For this review, take the finished solid that the model builds, in its own axes (mm). Face numbers are marked on the shaded views. A direction names the side the tool comes from. Round coordinates to 2 decimals unless told otherwise and drop trailing zeros. Loops run counter-clockwise (first coordinate to the right, second up) from the corner with the lowest first, then second, coordinate; pieces in that order, holes last. Notation, with made-up numbers: (75, 30.25) -> (133, 30.25) arc R9 ccw to (133, 38.25) -> close; hole circle Ø1 at (-35, 39.25). An arc over 180 degrees is marked (long way). One line per question, with ' | ' between items. Start each with the question number.
1. For the marked faces 1, 2 and 3, list the 3-axis set-ups (+Z, -Z, +X, -X, +Y, -Y) from which the entire face can be reached by the end or side of a thin tool; tool diameter is ignored.
2. Consider section A-A (y = 0). Write out the cut boundary in (x, z), and give its area (3 significant figures).
3. Consider section C-C (z = 233.5). Write out the cut boundary in (x, y).
4. For pin 1 Ø2.5 at (y, z) = (17.5, -3) entering from -X; pin 2 Ø4 at (y, z) = (26.5, 215.5) entering from +X (3 decimals); pin 3 Ø1 at (x, z) = (23.5, 280) entering from -Y, all flat-tipped, find the tip position at first contact; note any pin that passes through.
5. Wall thickness on line 1 along X through (y, z) = (19.5, 253); line 2 along Y through (x, z) = (-28, 194); line 3 along Z through (x, y) = (28, 15): over which ranges is each line inside the solid? List them lowest first.
6. Consider section B-B (x = 0). Write out the cut boundary in (y, z).
7. Consider section D-D (z = 160.5). Write out the cut boundary in (x, y).
```python
from build123d import *

# Parameters (mm, degrees)
BOSS_EXTRUDE1_DEPTH      = 400
BOSS_EXTRUDE1_DEPTH_BACK = 20
SKETCH1_R                = 25
CHAMFER1_SIZE            = 4
CUT_EXTRUDE1_DEPTH       = 10
SKETCH3_R                = 35
BOSS_EXTRUDE2_DEPTH      = 70
CHAMFER2_SIZE            = 2
CHAMFER3_SIZE            = 4


with BuildPart() as part:
    # Sketch1 → Boss-Extrude1 (new, two sides: drawn at the far end of the back side and taken through both)
    with BuildSketch(Plane.XY.offset(-BOSS_EXTRUDE1_DEPTH_BACK)):
        Circle(SKETCH1_R)
    extrude(amount=BOSS_EXTRUDE1_DEPTH + BOSS_EXTRUDE1_DEPTH_BACK)

    # Chamfer1
    chamfer1_edges = [part.edges().sort_by_distance(p)[0] for p in [
        (-25, 0, -20),
        (-25, 0, 400),
    ]]
    chamfer(chamfer1_edges, length=CHAMFER1_SIZE)

    # Sketch2 → Cut-Extrude1 (cut)
    with BuildSketch(Plane(origin=(0, 25, 0), x_dir=(1, 0, 0), z_dir=(0, 1, 0))):
        with BuildLine():
            Line((7.5, -15), (7.5, 55))
            Line((7.5, 55), (-7.5, 55))
            Line((-7.5, 55), (-7.5, -15))
            ThreePointArc((-7.5, -15), (0, -22.5), (7.5, -15))
        make_face()
    extrude(amount=-CUT_EXTRUDE1_DEPTH, mode=Mode.SUBTRACT)

    # Sketch3 → Boss-Extrude2 (add, symmetric)
    with BuildSketch(Plane.XY.offset(250)):
        Circle(SKETCH3_R)
    extrude(amount=BOSS_EXTRUDE2_DEPTH, both=True)

    # Chamfer2
    chamfer2_edges = [part.edges().sort_by_distance(p)[0] for p in [
        (-35, 0, 180),
        (-35, 0, 320),
    ]]
    chamfer(chamfer2_edges, length=CHAMFER2_SIZE)

    # Chamfer3
    chamfer3_edges = [part.edges().sort_by_distance(p)[0] for p in [
        (-25, 0, 320),
        (-25, 0, 180),
    ]]
    chamfer(chamfer3_edges, length=CHAMFER3_SIZE)


solid = part.part
```
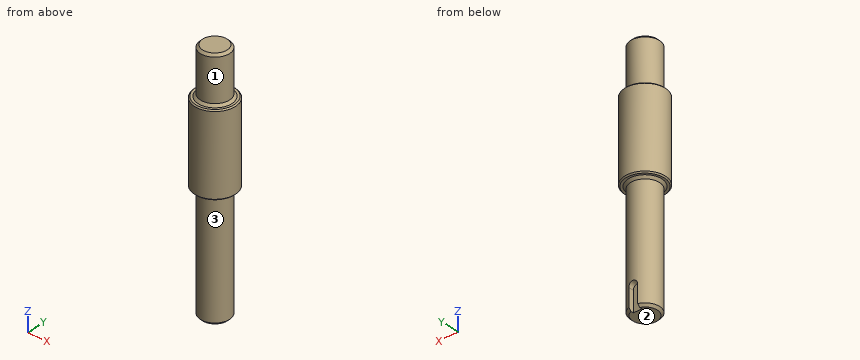
Answer block:
1) face 1: +Z | face 2: -Z, +X, -X, +Y, -Y | face 3: -Z
2) outline: (-35, 182) -> (-33, 180) -> (-29, 180) -> (-25, 176) -> (-25, -16) -> (-21, -20) -> (21, -20) -> (25, -16) -> (25, 176) -> (29, 180) -> (33, 180) -> (35, 182) -> (35, 318) -> (33, 320) -> (29, 320) -> (25, 324) -> (25, 396) -> (21, 400) -> (-21, 400) -> (-25, 396) -> (-25, 324) -> (-29, 320) -> (-33, 320) -> (-35, 318) -> close | area: 23,800 mm2
3) outline: circle Ø70 at (0, 0)
4) pin 1: stops at x = -19 | pin 2: stops at x = 24.995 | pin 3: stops at y = -26.38
5) line 1: x = -29.06 to 29.06 | line 2: y = -21 to 21 | line 3: z = 180 to 320
6) outline: (-35, 182) -> (-33, 180) -> (-29, 180) -> (-25, 176) -> (-25, -16) -> (-21, -20) -> (15, -20) -> (15, 22.5) -> (25, 22.5) -> (25, 176) -> (29, 180) -> (33, 180) -> (35, 182) -> (35, 318) -> (33, 320) -> (29, 320) -> (25, 324) -> (25, 396) -> (21, 400) -> (-21, 400) -> (-25, 396) -> (-25, 324) -> (-29, 320) -> (-33, 320) -> (-35, 318) -> close
7) outline: circle Ø50 at (0, 0)
